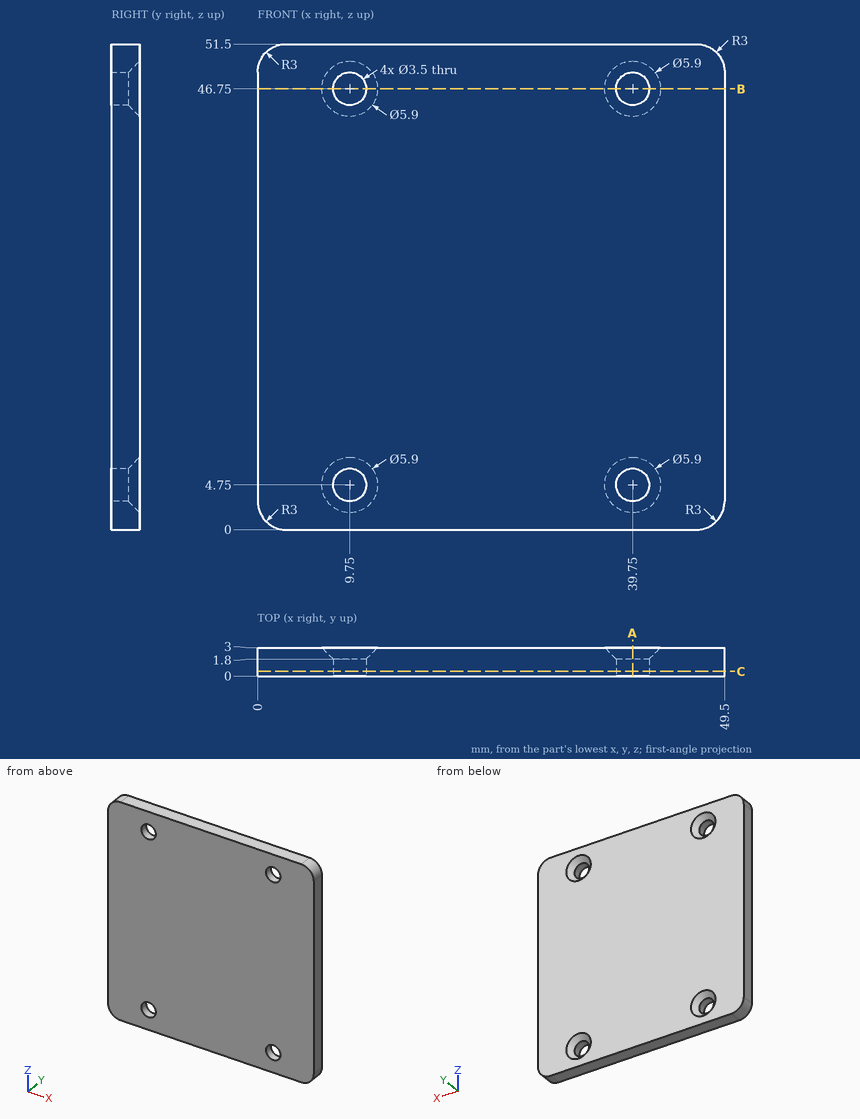
Could you check a few things on this drawing? It's one solid part, dimensions in mm from its lowest x, y, z. Give positions to 0.01 mm unless a question says otherwise; leave off trailing zeros. Order: outer loops, then holes, each group sorted by start corner. A loop starts at its lowest first (then second) coordinate and runs counter-clockwise, first axis right, second up. Notation, with made-up numbers: (-35.5, 1.25) - (-21.5, 1.25) arc R25 ccw to (-21.5, 34.25) - close; hole circle Ø1 at (-19, 84.25). An arc over 180 degrees is marked (long way). Return JSON: item names as keys, results as strings. Group by question number.
Q1. Suppose I cut it at B-B, the plane z = 46.75. Please give me the cut outline in (x, y), and give its area (3 significant figures).
Q2. Suppose I cut it at A-A, the plane x = 39.75. Please give me the cut outline in (y, z).
Q3. Please list where these lines run through material, in increasing order: line 1 along X through (y, z) = (0.85, 46.75); line 2 along Z through (x, y) = (38.5, 1.6); line 3 along X through (y, z) = (2.7, 4.5). Write a range as [from, to].
Q4. Suppose I cut it at C-C, the plane y = 0.5. Please give me the cut outline in (x, z).
Resolved:
{
 "1": {"outline": "(0, 0) - (8, 0) - (8, 1.8) - (6.8, 3) - (0, 3) - close; (11.5, 0) - (38, 0) - (38, 1.8) - (36.8, 3) - (12.7, 3) - (11.5, 1.8) - close; (41.5, 0) - (49.5, 0) - (49.5, 3) - (42.7, 3) - (41.5, 1.8) - close", "area": "125 mm2"},
 "2": {"outline": "(0, 0) - (3, 0) - (3, 1.8) - (1.8, 3) - (0, 3) - close; (0, 6.5) - (1.8, 6.5) - (3, 7.7) - (3, 43.8) - (1.8, 45) - (0, 45) - close; (0, 48.5) - (1.8, 48.5) - (3, 49.7) - (3, 51.5) - (0, 51.5) - close"},
 "3": {"line 1": "x = [0, 8], [11.5, 38], [41.5, 49.5]", "line 2": "z = [0, 3.53], [5.97, 45.53], [47.97, 51.5]", "line 3": "x = [0, 7.11], [12.39, 37.11], [42.39, 49.5]"},
 "4": {"outline": "(0, 3) arc R3 ccw to (3, 0) - (46.5, 0) arc R3 ccw to (49.5, 3) - (49.5, 48.5) arc R3 ccw to (46.5, 51.5) - (3, 51.5) arc R3 ccw to (0, 48.5) - close; hole circle Ø3.5 at (9.75, 4.75); hole circle Ø3.5 at (9.75, 46.75); hole circle Ø3.5 at (39.75, 4.75); hole circle Ø3.5 at (39.75, 46.75)"}
}
